Could you check a few things on this model? Use its own coordinates, in mm. Coordinates: 2 decimals unless noted, no trailing zeros. Loops run counter-clockwise (first coordinate to the right, second up) from the corner with the lowest first, then second, coordinate; pieces in that order, holes last. Notation, with made-up numbers: M 80.5,37 L 130.5,37 A23 cw 130.5,52 Z; hole C -9.75,39 d5. An arc over 180 degrees is marked long. Write each question's results on one line, items separated by ' | '.
```python
from build123d import *

# Parameters (mm, degrees)
EXTRUDE_1_DEPTH              = 12
HOLE_WIZARD_M6_1_D           = 5
HOLE_WIZARD_M6_1_DEPTH       = 15
HOLE_WIZARD_M6_1_CSINK_D     = 6.05
HOLE_WIZARD_M6_1_CSINK_ANGLE = 90
HOLE_WIZARD_M6_1_TIP         = 1.502151548
HOLE_WIZARD_M6_2_D           = 5
HOLE_WIZARD_M6_2_DEPTH       = 15
HOLE_WIZARD_M6_2_CSINK_D     = 6.05
HOLE_WIZARD_M6_2_CSINK_ANGLE = 90
HOLE_WIZARD_M6_2_TIP         = 1.502151548


with BuildPart() as part:
    # 草图1 → 凸台-拉伸1 (new body)
    with BuildSketch(Plane.XY):
        Polygon((0, 8.456375839), (0, 18.456375839), (50, 158.456375839), (60, 158.456375839), (60, 8.456375839), align=None)
    extrude(amount=EXTRUDE_1_DEPTH)

    # M6 螺纹孔1
    with Locations(Plane(origin=(0, 8.456375839, 0), x_dir=(-1, 0, 0), z_dir=(0, -1, 0))):
        with Locations((-50, -6), (-10, -6)):
            CounterSinkHole(HOLE_WIZARD_M6_1_D / 2, HOLE_WIZARD_M6_1_CSINK_D / 2, depth=HOLE_WIZARD_M6_1_DEPTH, counter_sink_angle=HOLE_WIZARD_M6_1_CSINK_ANGLE)
            with Locations((0, 0, -(HOLE_WIZARD_M6_1_DEPTH + HOLE_WIZARD_M6_1_TIP / 2))):  # 118° drill point
                Cone(0, HOLE_WIZARD_M6_1_D / 2, HOLE_WIZARD_M6_1_TIP, mode=Mode.SUBTRACT)

    # M6 螺纹孔2
    with Locations(Plane(origin=(60, 0, 0), x_dir=(0, 0, -1), z_dir=(1, 0, 0))):
        with Locations((-6, 33.456375839), (-6, 133.456375839)):
            CounterSinkHole(HOLE_WIZARD_M6_2_D / 2, HOLE_WIZARD_M6_2_CSINK_D / 2, depth=HOLE_WIZARD_M6_2_DEPTH, counter_sink_angle=HOLE_WIZARD_M6_2_CSINK_ANGLE)
            with Locations((0, 0, -(HOLE_WIZARD_M6_2_DEPTH + HOLE_WIZARD_M6_2_TIP / 2))):  # 118° drill point
                Cone(0, HOLE_WIZARD_M6_2_D / 2, HOLE_WIZARD_M6_2_TIP, mode=Mode.SUBTRACT)


solid = part.part
```
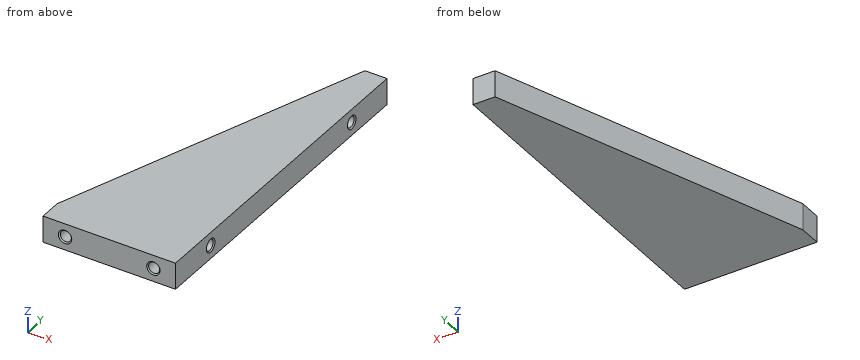
(1) Imagine slicing it at A-A, the plane y = 146. List the corners of the cut face in (x, z) for me, and give its area (3 significant figures).
Reported:
outline: M 45.55,0 L 60,0 L 60,12 L 45.55,12 Z | area: 173 mm2
(2) Please list where these lines run through material, in increasing order: probe 1 along Y at (x, z) = (56, 4); probe 2 along Y at (x, z) = (55, 6); probe 3 along Z at (x, y) = (10, 16.5). Write a range as from..to.
Reported:
probe 1: y = 8.46..31.96, 34.96..131.96, 134.96..158.46 | probe 2: y = 8.46..30.96, 35.96..130.96, 135.96..158.46 | probe 3: z = 0..3.5, 8.5..12
(3) Will this pin go through, and if not, where does the flat tip stop? P1, Ø4, axis at y = 133.46, z = 6, coming from the +X side.
Reported:
P1: stops at x = 44.7
(4) Imagine slicing it at B-B, the plane x = 23.5. List the corners of the cut face in (y, z) for me, and give its area (3 significant figures).
Reported:
outline: M 8.46,0 L 84.26,0 L 84.26,12 L 8.46,12 Z | area: 910 mm2
